from build123d import *

# Parameters (mm, degrees)
CHAMFER1_SIZE = 1


with BuildPart() as part:
    # Sketch1 → Revolve1 (revolve)
    with BuildSketch(Plane.XY, mode=Mode.PRIVATE) as revolve1_sk:
        with BuildLine():
            Line((-0.96339526, 77.991604501), (-5, 71))
            Line((-5, 71), (-5, 15))
            Line((-5, 15), (-8, 15))
            Line((-8, 15), (-8, 0))
            Line((-8, 0), (0, 0))
            Line((0, 0), (0, 78.491604501))
            Line((0, 78.491604501), (-0.097369856, 78.491604501))
            ThreePointArc((-0.097369856, 78.491604501), (-0.597369856, 78.357629904), (-0.96339526, 77.991604501))
        make_face()
    revolve(revolve1_sk.sketch.rotate(Axis((0, 0, 0), (0, 1, 0)), 270), axis=Axis((0, 0, 0), (0, 1, 0)))

    # Chamfer1
    chamfer1_edges = [part.edges().sort_by_distance(p)[0] for p in [
        (0, 0, 8),
        (0, 15, 8),
    ]]
    chamfer(chamfer1_edges, length=CHAMFER1_SIZE)


solid = part.part
The listing builds one solid part. Answer for the finished solid, in the listing's coordinates (mm). A direction names the side the tool comes from. Give positions to 0.01 mm unless a question says otherwise; leave off trailing zeros. Write each loop counter-clockwise with the first axis right and the second up, starting at its lowest first coordinate (ties: lowest second). Pieces come first, ordered by that corner, then holes. Notation, with made-up numbers: (82, 21.25) -> (100, 21.25) arc R12 cw to (100, 44.25) -> close; hole circle Ø7 at (6.5, 89.25). An arc over 180 degrees is marked (long way). Use a Markdown table: item, result.
(1) For faces 1 (the cylindrical face through (7.81, 7.41, 1.73)), 2 (the flat face through (-5, 15, -2)), determine the directions among +Z, -Z, +X, -X, +Y, -Y from which every point of the face is accessible in a straight line to the end or side of a thin tool.
Return value:
| item | result |
|---|---|
| face 1 | +Y, -Y |
| face 2 | +Y |
(2) Section A-A, the plane y = 28 is taken. Determine the outline of the cut face in (x, z), then the cut area to 3 significant figures.
Return value:
| item | result |
|---|---|
| outline | circle Ø10 at (0, 0) |
| area | 78.5 mm2 |
(3) Find the intervals of material crossed by probe 1 along Y at (x, z) = (-4.75, -1.75); probe 2 along Z at (x, y) = (-0.25, 52); probe 3 along Z at (x, y) = (-0.5, 5.5), in increasing order. Write a range as from..to.
Return value:
| item | result |
|---|---|
| probe 1 | 0..15 |
| probe 2 | -4.99..4.99 |
| probe 3 | -7.98..7.98 |
(4) Flat-ended cylindrical pins translate along their axes: P1, Ø3, axis at y = 47, z = 0.5, coming from the +X side; P2, Ø6, axis at y = 23, z = -3, coming from the -X side; P3, Ø1.5, axis at x = 6, y = 17.5, coming from the +Z side; P4, Ø4, axis at x = 1, z = -5, coming from the +Y side. Find the tip coordinate at first contact, or state that the pin passes through.
Return value:
| item | result |
|---|---|
| P1 | x = 5 |
| P2 | x = -5 |
| P3 | through |
| P4 | y = 74.29 |
